```python
from build123d import *

# Parameters (mm, degrees)
BASE_PLATE_SKETCH_W        = 86
BASE_PLATE_SKETCH_H        = 64
BASE_PLATE_86X64X10_DEPTH  = 10
UPPER_LAYER_SKETCH_W       = 86
UPPER_LAYER_SKETCH_H       = 64
UPPER_LAYER_BOSS_10_DEPTH  = 10
ANGLED_STEP_BOSS_19_DEPTH  = 19
ANGLED_CUT_25DEG_DEPTH     = 65
THROUGH_HOLE_SKETCH_R      = 7
THROUGH_HOLE_14_DEPTH      = 65
TRIANGULAR_NOTCH_CUT_DEPTH = 10
SIDE_BOSS_SKETCH_W         = 30
SIDE_BOSS_SKETCH_H         = 7
SIDE_BOSS_64_DEPTH         = 64
SIDE_BOSS_HOLE_SKETCH_R    = 7
SIDE_BOSS_HOLE_14_DEPTH    = 64


with BuildPart() as part:
    # Base Plate Sketch → Base Plate 86x64x10 (new body)
    with BuildSketch(Plane.XY):
        with Locations((43, 32)):
            Rectangle(BASE_PLATE_SKETCH_W, BASE_PLATE_SKETCH_H)
    extrude(amount=BASE_PLATE_86X64X10_DEPTH)

    # Upper Layer Sketch → Upper Layer Boss 10 (add)
    with BuildSketch(Plane.XY.offset(10)):
        with Locations((43, 32)):
            Rectangle(UPPER_LAYER_SKETCH_W, UPPER_LAYER_SKETCH_H)
    extrude(amount=UPPER_LAYER_BOSS_10_DEPTH)

    # Angled Step Sketch → Angled Step Boss 19 (add)
    with BuildSketch(Plane.XY.offset(20)):
        Polygon((54, 52), (54, 64), (0, 64), (0, 0), (10.366819179, 0), align=None)
    extrude(amount=ANGLED_STEP_BOSS_19_DEPTH)

    # Angled Cut Sketch → Angled Cut 25deg (cut)
    with BuildSketch(Plane.ZY):
        Polygon((39, 64), (39, 40), (27.808616204, 64), align=None)
    extrude(amount=-ANGLED_CUT_25DEG_DEPTH, mode=Mode.SUBTRACT)

    # Through Hole Sketch → Through Hole Ø14 (cut)
    with BuildSketch(Plane.XY.offset(20)):
        with Locations((46, 26)):
            Circle(THROUGH_HOLE_SKETCH_R)
    extrude(amount=-THROUGH_HOLE_14_DEPTH, mode=Mode.SUBTRACT)

    # Triangular Notch Sketch → Triangular Notch Cut (cut)
    with BuildSketch(Plane.XY.offset(20)):
        Polygon((86, 0), (86, 26), (64.183409589, 0), align=None)
    extrude(amount=-TRIANGULAR_NOTCH_CUT_DEPTH, mode=Mode.SUBTRACT)

    # Side Boss Sketch → Side Boss 64 (add)
    with BuildSketch(Plane.XZ):
        with Locations((46, -3.5)):
            Rectangle(SIDE_BOSS_SKETCH_W, SIDE_BOSS_SKETCH_H)
    extrude(amount=-SIDE_BOSS_64_DEPTH)

    # Side Boss Hole Sketch → Side Boss Hole Ø14 (cut)
    with BuildSketch(Plane.XY):
        with Locations((46, 26)):
            Circle(SIDE_BOSS_HOLE_SKETCH_R)
    extrude(amount=-SIDE_BOSS_HOLE_14_DEPTH, mode=Mode.SUBTRACT)


solid = part.part
```
Verification items for the finished model (mm, model axes). A direction names the side the tool comes from. Give positions to 0.01 mm unless a question says otherwise; leave off trailing zeros. Order: outer loops, then holes, each group sorted by start corner. A loop starts at its lowest first (then second) coordinate and runs counter-clockwise, first axis right, second up. Notation, with made-up numbers: (-39, 31.25) -> (-27, 31.25) arc R23 ccw to (-27, 49.25) -> close; hole circle Ø7 at (-27, 37). An arc over 180 degrees is marked (long way). One line per item, written item: value.
(1) Draft check along X on faces 1 (the face through (56, 25, 20)), 2 (the face through (54, 58, 25)), 3 (the face through (49.23, 19.79, 6.69)), 4 (the face through (0, 32, 19)). Enter one of: pulls with the +X half, pulls with the -X half, needs draft (parallel to the pull), parting line crosses it, or undercut.
Final values:
face 1: needs draft
face 2: pulls with the +X half
face 3: undercut
face 4: pulls with the -X half
(2) Sectioned sample at C-C on y = 27. Record the cut outline in (x, z), then the cut area to 3 significant figures.
Final values:
outline: (0, 0) -> (31, 0) -> (31, -7) -> (39.07, -7) -> (39.07, 20) -> (33.02, 20) -> (33.02, 39) -> (0, 39) -> close; (52.93, -7) -> (61, -7) -> (61, 0) -> (86, 0) -> (86, 20) -> (52.93, 20) -> close
area: 2,180 mm^2
(3) Scan lines: line 1 along Y through (x, z) = (46, 6); line 2 along Z through (x, y) = (50.5, 42); line 3 along Z through (x, y) = (12, 37). Record each from-to range of solid material in increasing order. Write a range as [from, to].
Final values:
line 1: [0, 19], [33, 64]
line 2: [-7, 20]
line 3: [0, 39]
(4) Sectioned sample at D-D on y = 54. Record the cut outline in (x, z).
Final values:
outline: (0, 0) -> (31, 0) -> (31, -7) -> (61, -7) -> (61, 0) -> (86, 0) -> (86, 20) -> (54, 20) -> (54, 32.47) -> (0, 32.47) -> close
(5) Sectioned sample at B-B on x = 46. Record the cut outline in (y, z).
Final values:
outline: (0, -7) -> (19, -7) -> (19, 20) -> (0, 20) -> close; (33, -7) -> (64, -7) -> (64, 27.81) -> (42.47, 37.85) -> (42.47, 20) -> (33, 20) -> close
(6) Gauge pin test, flat ends, axial feed: pin 1 (13 mm diameter, centred on y = 60.5, z = 28, fed in from +X); pin 2 (15.5 mm diameter, centred on x = 22, y = 41, fed in from -Z); pin 3 (3.5 mm diameter, centred on y = 45.5, z = -3, fed in from +X). Record the tip position at first contact, or that the pin passes through.
Final values:
pin 1: x = 54
pin 2: z = 0
pin 3: x = 61
(7) Tool access check on faces 5 (the face through (31, 32, -4)), 6 (the face through (61, 32, -4)), 7 (the face through (75.244, 13.182, 15.07)). Record the directions out of +Z, -Z, +X, -X, +Y, -Y that give a thin tool (end or side, any length) a straight path to the whole face; none if there is none.
Final values:
face 5: -Z, -X, +Y, -Y
face 6: -Z, +X, +Y, -Y
face 7: +Z, +X, -Y
(8) Sectioned sample at A-A on z = 2.5. Record the cut outline in (x, y), then the cut area to 3 significant figures.
Final values:
outline: (0, 0) -> (86, 0) -> (86, 64) -> (0, 64) -> close; hole circle Ø14 at (46, 26)
area: 5,350 mm^2
